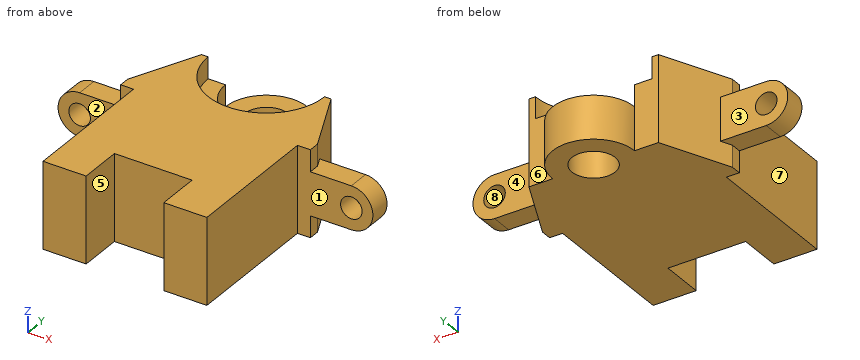
from build123d import *

# Parameters (mm, degrees)
PEDESTAL_BODY_DEPTH      = 20
FRONT_RECESS_54_SKETCH_R = 27
FRONT_RECESS_54_DEPTH    = 10
INNER_RECESS_38_SKETCH_R = 19
INNER_RECESS_38_DEPTH    = 10
HUB_38_SKETCH_R          = 19
HUB_38_DEPTH             = 20
BORE_20_SKETCH_R         = 10
BORE_20_DEPTH            = 100.523866484
MOUNTING_EAR_SKETCH_R    = 5
MOUNTING_EAR_DEPTH       = 10


with BuildPart() as part:
    # Pedestal Profile Sketch → Pedestal Body (new, symmetric)
    with BuildSketch(Plane.XY):
        Polygon((18, -32), (38, -32), (38, 32), (44, 32), (44, 37), (30, 68), (-30, 68), (-44, 37), (-44, 32), (-38, 32), (-38, -32), (-18, -32), (-18, -12), (18, -12), align=None)
    extrude(amount=PEDESTAL_BODY_DEPTH, both=True)

    # Front Recess Ø54 Sketch → Front Recess Ø54 (cut)
    with BuildSketch(Plane.XY.offset(20)):
        with Locations((0, 68)):
            Circle(FRONT_RECESS_54_SKETCH_R)
    extrude(amount=-FRONT_RECESS_54_DEPTH, mode=Mode.SUBTRACT)

    # Inner Recess Ø38 Sketch → Inner Recess Ø38 (cut)
    with BuildSketch(Plane.XY.offset(10)):
        with Locations((0, 68)):
            Circle(INNER_RECESS_38_SKETCH_R)
    extrude(amount=-INNER_RECESS_38_DEPTH, mode=Mode.SUBTRACT)

    # Hub Ø38 Sketch → Hub Ø38 (add)
    with BuildSketch(Plane.XY):
        with Locations((0, 68)):
            Circle(HUB_38_SKETCH_R)
    extrude(amount=-HUB_38_DEPTH)

    # Bore Ø20 Sketch → Bore Ø20 (cut, through all)
    with BuildSketch(Plane.XY):
        with Locations((0, 68)):
            Circle(BORE_20_SKETCH_R)
    extrude(amount=-BORE_20_DEPTH, mode=Mode.SUBTRACT)

    # Mounting Ear Sketch → Mounting Ear (add)
    with BuildSketch(Plane.XZ.offset(-32)):
        with BuildLine():
            Line((-63, 10), (-44, 10))
            Line((-44, 10), (-38, 10))
            Line((-38, 10), (-38, -10))
            Line((-38, -10), (-44, -10))
            Line((-44, -10), (-63, -10))
            ThreePointArc((-63, -10), (-73, 0), (-63, 10))
        make_face()
        with Locations(Location((-63, 0, 0), (0, 0, 270))):
            Circle(MOUNTING_EAR_SKETCH_R, mode=Mode.SUBTRACT)
    mounting_ear = extrude(amount=-MOUNTING_EAR_DEPTH)

    # Mounting Ear Mirror: Mounting Ear across plane
    add(mounting_ear.mirror(Plane(origin=(0, 0, 0), x_dir=(0, 0, 1), z_dir=(1, 0, 0))))


solid = part.part
Check sheet for the modelled part. Datum: model origin and axes. Units: mm. Face numbers are marked on the shaded views. A direction names the side the tool comes from. Round coordinates to 2 decimals unless told otherwise and drop trailing zeros. Loops run counter-clockwise (first coordinate to the right, second up) from the corner with the lowest first, then second, coordinate; pieces in that order, holes last. Notation, with made-up numbers: (29, 22.5) - (77, 22.5) arc R7 ccw to (77, 31.5) - close; hole circle Ø3 at (16, 66.5). An arc over 180 degrees is marked (long way). Answer as CSV lines item,"result". Start each with the question number.
Item 1: Release check for a two-part mould opening along X. For the marked faces 6, 7 and 8 record: +X half, -X half, draft (parallel to the pull), parting line (faces both ways), or undercut.
Item 2: Set-up check for the marked faces 1, 2, 3, 4 and 5: record each of +Z, -Z, +X, -X, +Y, -Y from which the full face is reachable in a straight line by a thin tool's end or side.
Item 3: Section check D-D (z = 2). Record the boundary of the cut face in (x, y), and give its area (3 significant figures).
Item 4: Section check C-C (y = 70). Record the boundary of the cut face in (x, z).
Item 5: Depth check by flat-ended pin: P1, Ø11.5, axis at x = -63, z = 0, coming from the -Y side; P2, Ø1, axis at y = -7.5, z = -13.5, coming from the +X side; P3, Ø13.5, axis at x = -9, y = 60.5, coming from the +Z side. Enter the tip coordinate at first touch or a pass-through.
Item 6: Section check B-B (z = -15). Record the boundary of the cut face in (x, y).
Item 7: Scan lines: line 1 (X direction, y = 36, z = 0); line 2 (Z direction, x = 63, y = 36.75); line 3 (X direction, y = -23, z = -2). Record each from-to range of solid material in increasing order. Write a range as [from, to].
Item 8: Section check A-A (x = 0). Record the boundary of the cut face in (y, z), and give its area (3 significant figures).
Report:
1,face 6,"draft"
1,face 7,"-X half"
1,face 8,"undercut"
2,face 1,"+Z, -Z, +X, -Y"
2,face 2,"+Z, -Z, -X, -Y"
2,face 3,"+Z, -Z, -X, +Y"
2,face 4,"+Z, -Z, +X, +Y"
2,face 5,"+Z, -Z, -Y"
3,outline,"(-72.8, 32) - (-67.58, 32) - (-67.58, 42) - (-72.8, 42) - close; (-58.42, 32) - (-38, 32) - (-38, -32) - (-18, -32) - (-18, -12) - (18, -12) - (18, -32) - (38, -32) - (38, 32) - (58.42, 32) - (58.42, 42) - (41.74, 42) - (30, 68) - (19, 68) arc R19 cw to (-19, 68) - (-30, 68) - (-41.74, 42) - (-58.42, 42) - close; (67.58, 32) - (72.8, 32) - (72.8, 42) - (67.58, 42) - close"
3,area,"6,710 mm2"
4,outline,"(-18.89, -20) - (-9.8, -20) - (-9.8, 0) - (-18.89, 0) - close; (9.8, -20) - (18.89, -20) - (18.89, 0) - (9.8, 0) - close"
5,P1,"stops at y = 32"
5,P2,"stops at x = 38"
5,P3,"stops at z = 0"
6,outline,"(-44, 32) - (-38, 32) - (-38, -32) - (-18, -32) - (-18, -12) - (18, -12) - (18, -32) - (38, -32) - (38, 32) - (44, 32) - (44, 37) - (30, 68) - (19, 68) arc R19 ccw to (-19, 68) - (-30, 68) - (-44, 37) - close; hole circle Ø20 at (0, 68)"
7,line 1,"x = [-73, -68], [-58, 58], [68, 73]"
7,line 2,"z = [-10, -5], [5, 10]"
7,line 3,"x = [-38, -18], [18, 38]"
8,outline,"(-12, -20) - (58, -20) - (58, 0) - (49, 0) - (49, 10) - (41, 10) - (41, 20) - (-12, 20) - close; (78, -20) - (87, -20) - (87, 0) - (78, 0) - close"
8,area,"2,720 mm2"
